Model file for the job. Use its own axes, mm. Coordinates: 2 decimals unless noted, no trailing zeros. Return JSON: item names as keys, results as strings. Group by question number.
1) Flat gauge pins, fed straight in: pin 1 (4.5 mm diameter, centred on y = -22, z = 401, fed in from -X); pin 2 (2 mm diameter, centred on x = -10.5, z = 84, fed in from +Y). Where does each tip first touch, or does it go through?
2) Cut at A-A (z = 109.5). State how many separate pieces and enclosed holes the cut face has, and give its area (3 significant figures).
3) Probe line 1 (X direction, y = 17, z = 156); line 2 (Y direction, x = -16, z = 563); line 3 (Y direction, x = -3.5, z = 240.5). List the from-to ranges inside material, lowest first.
from build123d import *

# Parameters (mm, degrees)
SKETCH_1_R      = 3
EXTRUDE_1_DEPTH = 690


with BuildPart() as part:
    # 草图1 → 凸台-拉伸1 (new body)
    with BuildSketch(Plane.XY):
        Polygon((-27.495741056, 11.192504259), (-24.995741056, 11.192504259), (-24.995741056, 13.192504259), (-19.495741056, 13.192504259), (-19.495741056, 11.192504259), (-16.995741056, 11.192504259), (-16.995741056, 5.692504259), (-19.495741056, 5.692504259), (-19.495741056, 3.692504259), (-24.995741056, 3.692504259), (-24.995741056, 5.692504259), (-27.495741056, 5.692504259), (-27.495741056, -19.607495741), (-24.995741056, -19.607495741), (-24.995741056, -17.607495741), (-19.495741056, -17.607495741), (-19.495741056, -19.607495741), (-16.995741056, -19.607495741), (-16.995741056, -25.107495741), (-19.495741056, -25.107495741), (-19.495741056, -27.107495741), (-24.995741056, -27.107495741), (-24.995741056, -25.107495741), (-27.495741056, -25.107495741), (-27.495741056, -36.957495741), (-15.645741056, -36.957495741), (-15.645741056, -34.457495741), (-17.645741056, -34.457495741), (-17.645741056, -28.957495741), (-15.748076247, -28.957495741), (-15.748076247, -27.422563567), (-9.243405866, -27.422563567), (-9.243405866, -28.957495741), (-7.345741056, -28.957495741), (-7.345741056, -34.457495741), (-9.345741056, -34.457495741), (-9.345741056, -36.957495741), (2.504258944, -36.957495741), (2.504258944, -25.107495741), (0.004258944, -25.107495741), (0.004258944, -27.107495741), (-5.495741056, -27.107495741), (-5.495741056, -25.107495741), (-7.995741056, -25.107495741), (-7.995741056, -19.607495741), (-5.495741056, -19.607495741), (-5.495741056, -17.607495741), (0.004258944, -17.607495741), (0.004258944, -19.607495741), (2.504258944, -19.607495741), (2.504258944, 5.692504259), (0.004258944, 5.692504259), (0.004258944, 3.692504259), (-5.495741056, 3.692504259), (-5.495741056, 5.692504259), (-7.995741056, 5.692504259), (-7.995741056, 11.192504259), (-5.495741056, 11.192504259), (-5.495741056, 13.192504259), (0.004258944, 13.192504259), (0.004258944, 11.192504259), (2.504258944, 11.192504259), (2.504258944, 23.042504259), (-9.345741056, 23.042504259), (-9.345741056, 20.542504259), (-7.345741056, 20.542504259), (-7.345741056, 15.042504259), (-9.243405866, 15.042504259), (-9.243405866, 13.507572085), (-15.748076247, 13.507572085), (-15.748076247, 15.042504259), (-17.645741056, 15.042504259), (-17.645741056, 20.542504259), (-15.645741056, 20.542504259), (-15.645741056, 23.042504259), (-27.495741056, 23.042504259), align=None)
        with Locations((-21.995741056, 17.542504259)):
            Circle(SKETCH_1_R, mode=Mode.SUBTRACT)
        with Locations(Location((-2.995741056, 17.542504259, 0), (0, 0, 180))):
            Circle(SKETCH_1_R, mode=Mode.SUBTRACT)
        with Locations((-2.995741056, -31.457495741)):
            Circle(SKETCH_1_R, mode=Mode.SUBTRACT)
        with Locations(Location((-21.995741056, -31.457495741, 0), (0, 0, 180))):
            Circle(SKETCH_1_R, mode=Mode.SUBTRACT)
    extrude(amount=EXTRUDE_1_DEPTH)


solid = part.part
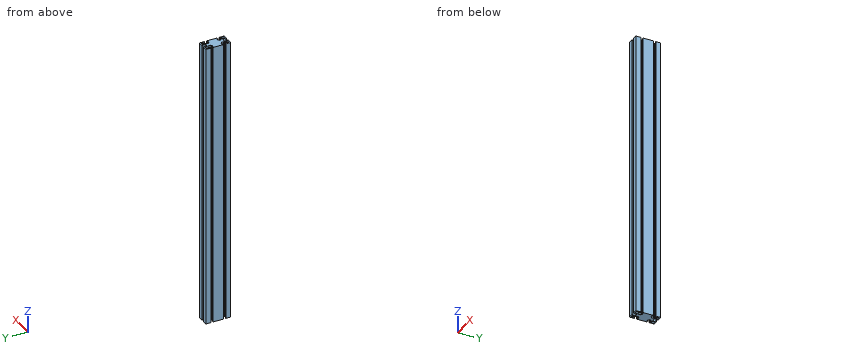
Answers below:
{
 "1": {"pin 1": "stops at x = -17", "pin 2": "stops at y = 13.51"},
 "2": {"separate pieces": "1", "enclosed holes": "4", "area": "1,200 mm^2"},
 "3": {"line 1": "x = -27.5 to -24.95, -19.05 to -17.65, -7.35 to -5.95, -0.05 to 2.5", "line 2": "y = -36.96 to -34.46, -28.96 to 15.04, 20.54 to 23.04", "line 3": "y = -36.96 to -34.41, -28.5 to -27.11, -17.61 to 3.69, 13.19 to 14.59, 20.5 to 23.04"}
}
